Job drawing, mm, ordinate dimensions from the low corner. One solid piece. A direction names the side the tool comes from. Round coordinates to 2 decimals unless told otherwise and drop trailing zeros. Loops run counter-clockwise (first coordinate to the right, second up) from the corner with the lowest first, then second, coordinate; pieces in that order, holes last.
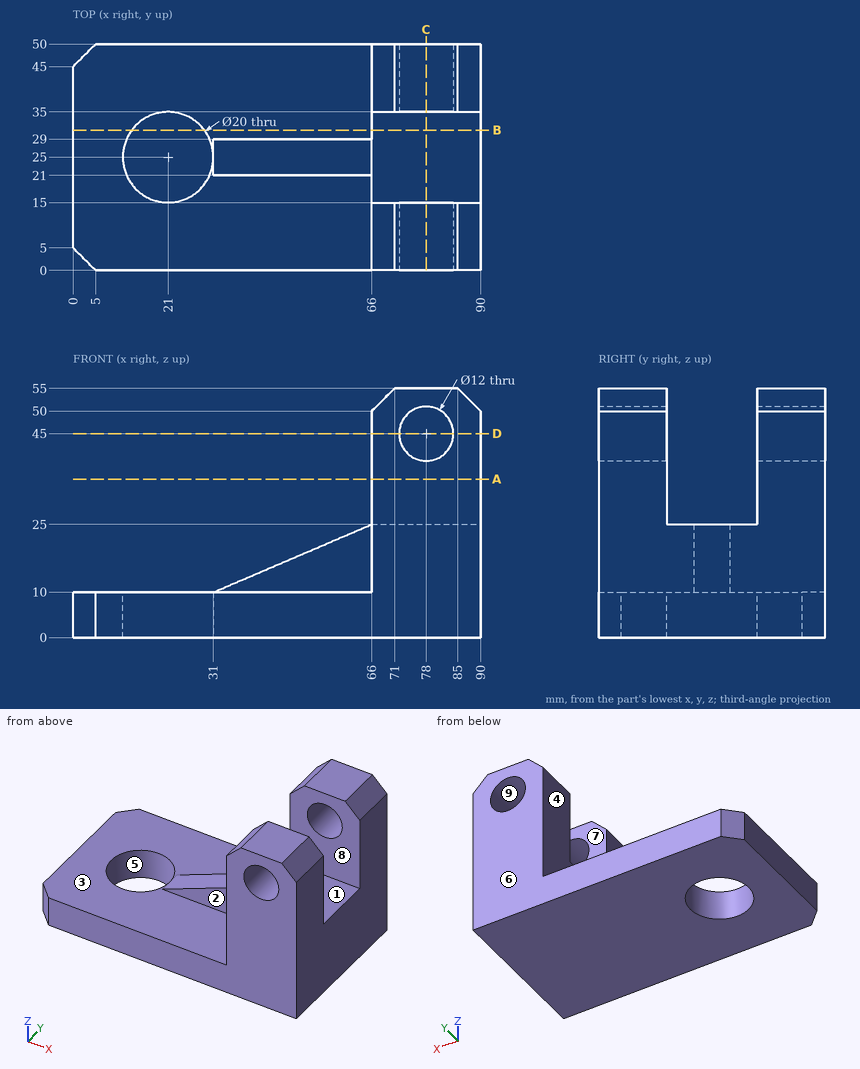
1) Drop flat-ended pins along their axis: pin 1 Ø6.5 at (y, z) = (9.5, 27) entering from -X; pin 2 Ø15 at (x, y) = (35, 30.5) entering from +Z; pin 3 Ø12 at (x, z) = (46.5, 16.5) entering from +Y; pin 4 Ø18 at (x, y) = (21, 25) entering from +Z. Give the stop position or say it passes through.
Values:
pin 1: stops at x = 66
pin 2: stops at z = 14.86
pin 3: stops at y = 29
pin 4: passes through
2) Mould opens along Y. For the marked faces 6, 7, 8 and 9 say: released by +Y, released by -Y, zero draft, split by the parting line, or undercut.
Values:
face 6: released by +Y
face 7: undercut
face 8: undercut
face 9: zero draft
3) Wall check: line 1 along X through (y, z) = (12, 45); line 2 along Z through (x, y) = (27.5, 38); line 3 along X through (y, z) = (4, 12). Give the ranges that are in metal, low to high.
Values:
line 1: x = 66 to 72, 84 to 90
line 2: z = 0 to 10
line 3: x = 66 to 90
4) Tool access for the marked faces 1, 2, 3, 4 and 5: list every direction of +Z, -Z, +X, -X, +Y, -Y with a clear straight run to the whole face (end or side of a thin tool).
Values:
face 1: +Z, +X, -X
face 2: +Z, -X, -Y
face 3: +Z, -X
face 4: +Z, -X, +Y
face 5: +Z, -Z
5) Slice it at B-B, the plane y = 31. Give the cut face in (x, z), then the cut area to 3 significant figures.
Values:
outline: (0, 0) - (13, 0) - (13, 10) - (0, 10) - close; (29, 0) - (90, 0) - (90, 25) - (66, 25) - (66, 10) - (29, 10) - close
area: 1,100 mm2
6) Slice it at D-D, the plane z = 45. Give the cut face in (x, y), then the cut area to 3 significant figures.
Values:
outline: (66, 0) - (72, 0) - (72, 15) - (66, 15) - close; (66, 35) - (72, 35) - (72, 50) - (66, 50) - close; (84, 0) - (90, 0) - (90, 15) - (84, 15) - close; (84, 35) - (90, 35) - (90, 50) - (84, 50) - close
area: 360 mm2
7) Slice it at C-C, the plane x = 78. Give the cut face in (y, z).
Values:
outline: (0, 0) - (50, 0) - (50, 39) - (35, 39) - (35, 25) - (15, 25) - (15, 39) - (0, 39) - close; (0, 51) - (15, 51) - (15, 55) - (0, 55) - close; (35, 51) - (50, 51) - (50, 55) - (35, 55) - close
8) Slice it at A-A, the plane z = 35. Give the cut face in (x, y), then the cut area to 3 significant figures.
Values:
outline: (66, 0) - (90, 0) - (90, 15) - (66, 15) - close; (66, 35) - (90, 35) - (90, 50) - (66, 50) - close
area: 720 mm2
